from build123d import *

# Parameters (mm, degrees)
SKETCH_1_R      = 25
EXTRUDE_1_DEPTH = 6
SKETCH_2_R      = 12.5
SKETCH_2_R_2    = 11
EXTRUDE_2_DEPTH = 8
SKETCH_3_R      = 5
EXTRUDE_3_DEPTH = 20
SKETCH_5_R      = 11.5
SKETCH_5_R_2    = 10.475
EXTRUDE_4_DEPTH = 4
SKETCH_6_R      = 1.425
EXTRUDE_5_DEPTH = 10


with BuildPart() as part:
    # 草图1 → 凸台-拉伸1 (new body)
    with BuildSketch(Plane.XY):
        Circle(SKETCH_1_R)
    extrude(amount=EXTRUDE_1_DEPTH)

    # 草图2 → 凸台-拉伸2 (add)
    with BuildSketch(Plane.XY.offset(6)):
        Circle(SKETCH_2_R)
        Circle(SKETCH_2_R_2, mode=Mode.SUBTRACT)
    extrude(amount=EXTRUDE_2_DEPTH)

    # 草图3 → 凸台-拉伸3 (add)
    with BuildSketch(Plane.XY.offset(6)):
        Circle(SKETCH_3_R)
    extrude(amount=EXTRUDE_3_DEPTH)

    # 草图5 → 凸台-拉伸4 (add)
    with BuildSketch(Plane(origin=(0, 0, 0), x_dir=(-1, 0, 0), z_dir=(0, 0, -1))):
        with Locations(Location((0, 0, 0), (0, 0, 180))):
            Circle(SKETCH_5_R)
        Circle(SKETCH_5_R_2, mode=Mode.SUBTRACT)
    extrude(amount=EXTRUDE_4_DEPTH)

    # 草图6 → 凸台-拉伸5 (add)
    with BuildSketch(Plane(origin=(0, 0, 0), x_dir=(-1, 0, 0), z_dir=(0, 0, -1))):
        with Locations(Location((0, 0, 0), (0, 0, 180))):
            Circle(SKETCH_6_R)
    extrude(amount=EXTRUDE_5_DEPTH)


solid = part.part
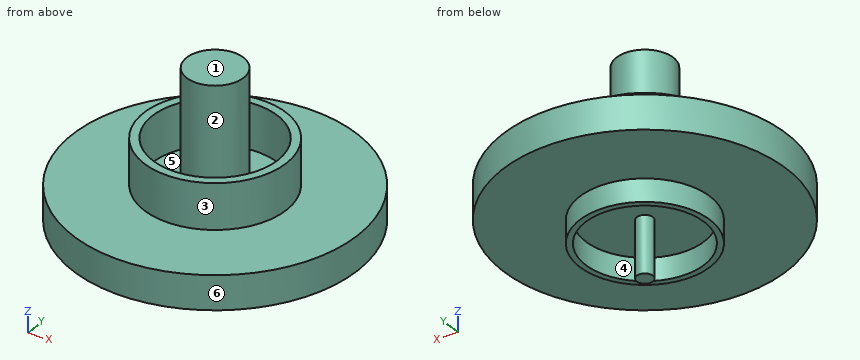
Could you check a few things on this model? Use its own coordinates, in mm. Face numbers are marked on the shaded views. A direction names the side the tool comes from. Give positions to 0.01 mm unless a question says otherwise; leave off trailing zeros. Order: outer loops, then holes, each group sorted by start corner. A loop starts at its lowest first (then second) coordinate and runs counter-clockwise, first axis right, second up.
1. I need wall thicknesses on L1, parallel to Y at x = 0, z = 12; L2, parallel to Y at x = 0, z = -0.9 (3 decimals); L3, parallel to Z at x = -11, y = 16. Which ranges of each line are inside material? Lowest first, please.
2. For the marked faces 4, 5 and 6, which set-ups out of +Z, -Z, +X, -X, +Y, -Y let a thin tool reach every point of the face, with its end or its side?
3. We'd pull the mould along X, two halves only. Please class the marked faces 1, 2 and 3: pulls with the +X half, pulls with the -X half, needs draft (parallel to the pull), parting line crosses it, or undercut.
4. Suppose I cut it at D-D (z = 4.5). List the corners of the cut face in (x, y) for me, plus the area to 3 significant figures.
5. Suppose I cut it at A-A (y = 0). List the corners of the cut face in (x, z) for me (3 decimals), plus the area to 3 significant figures.
6. Suppose I cut it at B-B (z = -2). List the corners of the cut face in (x, y) for me (3 decimals), plus the area to 3 significant figures.
7. Will these pins go through, and if not, where does the flat tip stop? P1, Ø2, axis at x = -9, z = -2, coming from the +Y side; P2, Ø18.5, axis at x = 2, y = 3.5, coming from the -Z side; P3, Ø1.5, axis at x = -13, y = 6, coming from the -Z side; P4, Ø6, axis at x = -11, y = -2.5, coming from the +Z side.
Solved:
1. L1: y = -12.5 to -11, -5 to 5, 11 to 12.5
1. L2: y = -11.5 to -10.475, -1.425 to 1.425, 10.475 to 11.5
1. L3: z = 0 to 6
2. face 4: -Z
2. face 5: +Z
2. face 6: +Z, -Z
3. face 1: needs draft
3. face 2: undercut
3. face 3: parting line crosses it
4. outline: circle Ø50 at (0, 0)
4. area: 1,960 mm2
5. outline: (-25, 0) - (-11.5, 0) - (-11.5, -4) - (-10.475, -4) - (-10.475, 0) - (-1.425, 0) - (-1.425, -10) - (1.425, -10) - (1.425, 0) - (10.475, 0) - (10.475, -4) - (11.5, -4) - (11.5, 0) - (25, 0) - (25, 6) - (12.5, 6) - (12.5, 14) - (11, 14) - (11, 6) - (5, 6) - (5, 26) - (-5, 26) - (-5, 6) - (-11, 6) - (-11, 14) - (-12.5, 14) - (-12.5, 6) - (-25, 6) - close
5. area: 561 mm2
6. outline: circle Ø23 at (0, 0); circle Ø2.85 at (0, 0); hole circle Ø20.95 at (0, 0)
6. area: 77.1 mm2
7. P1: stops at y = 8.26
7. P2: stops at z = -10
7. P3: stops at z = 0
7. P4: stops at z = 14
